Check sheet for the modelled part. Datum: model origin and axes. Units: mm. Face numbers are marked on the shaded views. A direction names the side the tool comes from. Round coordinates to 2 decimals unless told otherwise and drop trailing zeros. Order: outer loops, then holes, each group sorted by start corner. A loop starts at its lowest first (then second) coordinate and runs counter-clockwise, first axis right, second up. Notation, with made-up numbers: M -11,76 L 19,76 A24 cw 19,115 Z; hole C 76,55.25 d5. An arc over 180 degrees is marked long. One line per item, written item: value. Start each with the question number.
(1) Depth check by flat-ended pin: pin 1 Ø13 at (y, z) = (25.5, -25.5) entering from +X; pin 2 Ø6 at (y, z) = (45, -38.5) entering from -X; pin 3 Ø8 at (y, z) = (22.63, 22.63) entering from +X. Enter the tip coordinate at first touch or a pass-through.
(2) Cross-section at A-A, the plane z = 0. Count the separate pieces of the cut face and the enclosed holes in it, and give its area (4 significant figures).
(3) Thickness scan on L1, parallel to Y at x = 88.5, z = 0; L2, parallel to X at y = -23, z = 13.5; L3, parallel to Z at x = 90, y = -31.5. Record the ranges inside material, lowest first.
(4) Access from +Z, -Z, +X, -X, +Y, -Y to the whole of each face (thin tool, end or side, straight path). Record for the marked faces 1, 2 and 3.
(5) Cross-section at D-D, the plane z = -54. Enter the section's corners in (x, y), and give its area (3 significant figures).
(6) Cross-section at C-C, the plane y = -56. Enter the section's corners in (x, z).
(7) Release check for a two-part mould opening along Y. For the marked faces 4 and 5 record: released by +Y, released by -Y, zero draft, split by the parting line, or undercut.
from build123d import *

# Parameters (mm, degrees)
SKETCH2_R           = 3.5
CUT_EXTRUDE1_DEPTH  = 27
SKETCH3_R           = 5.5
CUT_EXTRUDE2_DEPTH  = 6
CIRPATTERN1_COUNT   = 4
CHAMFER1_SIZE       = 1
SKETCH4_R           = 52.910606105
CUT_EXTRUDE3_DEPTH  = 128
SKETCH5_R           = 67
BOSS_EXTRUDE1_DEPTH = 14
SKETCH6_R           = 19
BOSS_EXTRUDE2_DEPTH = 5
SKETCH7_R           = 3
SKETCH7_R_2         = 3.5
CUT_EXTRUDE4_DEPTH  = 41
SKETCH8_R           = 6
CUT_EXTRUDE5_DEPTH  = 6
CHAMFER2_SIZE       = 1
SKETCH9_R           = 7
CUT_EXTRUDE6_DEPTH  = 41
CIRPATTERN2_COUNT   = 4


with BuildPart() as part:
    # Sketch1 → Revolve1 (revolve)
    with BuildSketch(Plane.XY, mode=Mode.PRIVATE) as revolve1_sk:
        Polygon((0, 0), (0, 8), (75, 8), (75, 17.5), (82, 17.5), (82, 34), (92, 34), (92, 15), (120, 15), (120, 12), (207, 12), (207, 0), align=None)
    revolve(revolve1_sk.sketch.rotate(Axis((0, 0, 0), (1, 0, 0)), 90), axis=Axis((0, 0, 0), (1, 0, 0)))

    # Sketch2 → Cut-Extrude1 (cut)
    with BuildSketch(Plane(origin=(92, 0, 0), x_dir=(0, 0, -1), z_dir=(1, 0, 0))):
        with Locations((0, 24.5)):
            Circle(SKETCH2_R)
    cut_extrude1 = extrude(amount=-CUT_EXTRUDE1_DEPTH, mode=Mode.SUBTRACT)

    # Sketch3 → Cut-Extrude2 (cut)
    with BuildSketch(Plane.ZY.offset(-82)):
        with Locations((0, 24.5)):
            Circle(SKETCH3_R)
    cut_extrude2 = extrude(amount=-CUT_EXTRUDE2_DEPTH, mode=Mode.SUBTRACT)

    # CirPattern1: Cut-Extrude1, Cut-Extrude2 ×4 about axis
    cirpattern1_axis = Axis((0, 0, 0), (1, 0, 0))
    add([cut_extrude1.rotate(cirpattern1_axis, i * 360 / CIRPATTERN1_COUNT) for i in range(1, CIRPATTERN1_COUNT)], mode=Mode.SUBTRACT)
    add([cut_extrude2.rotate(cirpattern1_axis, i * 360 / CIRPATTERN1_COUNT) for i in range(1, CIRPATTERN1_COUNT)], mode=Mode.SUBTRACT)

    # Chamfer1
    chamfer1_edges = [part.edges().sort_by_distance(p)[0] for p in [
        (82, 0, -34),
        (75, 0, -17.5),
        (75, 0, -8),
        (0, 0, -8),
        (207, 0, -12),
        (120, 0, -15),
    ]]
    chamfer(chamfer1_edges, length=CHAMFER1_SIZE)

    # Sketch4 → Cut-Extrude3 (cut)
    with BuildSketch(Plane(origin=(92, 0, 0), x_dir=(0, 0, -1), z_dir=(1, 0, 0))):
        Circle(SKETCH4_R)
    extrude(amount=-CUT_EXTRUDE3_DEPTH, mode=Mode.SUBTRACT)

    # Sketch5 → Boss-Extrude1 (add)
    with BuildSketch(Plane.ZY.offset(-92)):
        Circle(SKETCH5_R)
    extrude(amount=BOSS_EXTRUDE1_DEPTH)

    # Sketch6 → Boss-Extrude2 (add)
    with BuildSketch(Plane.ZY.offset(-78)):
        Circle(SKETCH6_R)
    extrude(amount=BOSS_EXTRUDE2_DEPTH)

    # Sketch7 → Cut-Extrude4 (cut)
    with BuildSketch(Plane.ZY.offset(-78)):
        with Locations((0, -32)):
            Circle(SKETCH7_R)
        with Locations((22.627416998, 22.627416998)):
            Circle(SKETCH7_R_2)
        with Locations((22.627416998, -22.627416998)):
            Circle(SKETCH7_R_2)
        with Locations((-22.627416998, -22.627416998)):
            Circle(SKETCH7_R_2)
        with Locations((-22.627416998, 22.627416998)):
            Circle(SKETCH7_R_2)
    extrude(amount=-CUT_EXTRUDE4_DEPTH, mode=Mode.SUBTRACT)

    # Sketch8 → Cut-Extrude5 (cut)
    with BuildSketch(Plane(origin=(92, 0, 0), x_dir=(0, 0, -1), z_dir=(1, 0, 0))):
        with Locations((22.627416998, 22.627416998)):
            Circle(SKETCH8_R)
        with Locations((22.627416998, -22.627416998)):
            Circle(SKETCH8_R)
        with Locations((-22.627416998, -22.627416998)):
            Circle(SKETCH8_R)
        with Locations((-22.627416998, 22.627416998)):
            Circle(SKETCH8_R)
    extrude(amount=-CUT_EXTRUDE5_DEPTH, mode=Mode.SUBTRACT)

    # Chamfer2
    chamfer2_edges = [part.edges().sort_by_distance(p)[0] for p in [
        (73, 0, -19),
    ]]
    chamfer(chamfer2_edges, length=CHAMFER2_SIZE)

    # Sketch9 → Cut-Extrude6 (cut)
    with BuildSketch(Plane.ZY.offset(-78)):
        with Locations((0, -54)):
            Circle(SKETCH9_R)
    cut_extrude6 = extrude(amount=-CUT_EXTRUDE6_DEPTH, mode=Mode.SUBTRACT)

    # CirPattern2: Cut-Extrude6 ×4 about axis
    cirpattern2_axis = Axis((0, 0, 0), (1, 0, 0))
    for i in range(1, CIRPATTERN2_COUNT):
        add(cut_extrude6.rotate(cirpattern2_axis, i * 360 / CIRPATTERN2_COUNT), mode=Mode.SUBTRACT)


solid = part.part
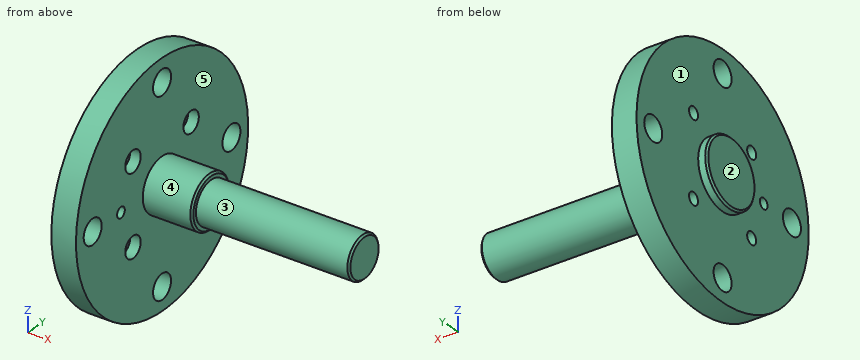
Values found:
1. pin 1: x = 92
1. pin 2: x = 78
1. pin 3: x = 86
2. separate pieces: 4
2. enclosed holes: 0
2. area: 4,515 mm^2
3. L1: -67 to -61, -47 to -35, -29 to 47, 61 to 67
3. L2: 78 to 92
3. L3: -59.13 to -2.96, 2.96 to 59.13
4. face 1: -X
4. face 2: +Z, -Z, -X, +Y, -Y
4. face 3: +X
5. outline: M 78,-39.66 L 92,-39.66 L 92,-7 L 78,-7 Z; M 78,7 L 92,7 L 92,39.66 L 78,39.66 Z
5. area: 915 mm^2
6. outline: M 78,-36.78 L 92,-36.78 L 92,-6.71 L 78,-6.71 Z; M 78,6.71 L 92,6.71 L 92,36.78 L 78,36.78 Z
7. face 4: split by the parting line
7. face 5: zero draft
